Could you check a few things on this model? Use its own coordinates, in mm. Face numbers are marked on the shaded views. A direction names the side the tool comes from. Give positions to 0.01 mm unless a question says otherwise; leave off trailing zeros. Order: outer loops, then holes, each group sorted by start corner. A loop starts at its lowest first (then second) coordinate and runs counter-clockwise, first axis right, second up. Notation, with made-up numbers: (40, 80) -> (81, 80) arc R10 ccw to (81, 90) -> close; hole circle Ø5 at (12, 37). An arc over 180 degrees is marked (long way). One line per item, written item: value.
```python
from build123d import *

# Parameters (mm, degrees)
CUT_EXTRUDE_3_DEPTH = 1
SKETCH_5_R          = 1.5
CUT_EXTRUDE_4_DEPTH = 10
CHAMFER_1_SIZE      = 0.5
CHAMFER_2_SIZE      = 0.5


with BuildPart() as part:
    # 草图1 → 旋转2 (revolve)
    with BuildSketch(Plane.XY, mode=Mode.PRIVATE) as revolve_2_sk:
        Polygon((-23.267570956, 0), (-23.267570956, 4), (-8.267570956, 4), (-8.267570956, 5), (-2.267570956, 5), (-2.267570956, 6.5), (0.732429044, 6.5), (0.732429044, 5), (10.732429044, 5), (10.732429044, 4), (18.732429044, 4), (18.732429044, 0), align=None)
    revolve(revolve_2_sk.sketch.rotate(Axis((-82.03072058, 0, 0), (1, 0, 0)), 90), axis=Axis((-82.03072058, 0, 0), (1, 0, 0)))

    # 草图4 → 切除-拉伸3 (cut)
    with BuildSketch(Plane(origin=(0, 4, 0), x_dir=(1, 0, 0), z_dir=(0, 1, 0))):
        with BuildLine():
            Line((-19.767570956, 1), (-11.767570956, 1))
            ThreePointArc((-11.767570956, 1), (-10.767570956, 0), (-11.767570956, -1))
            Line((-11.767570956, -1), (-19.767570956, -1))
            ThreePointArc((-19.767570956, -1), (-20.767570956, 0), (-19.767570956, 1))
        make_face()
    extrude(amount=-CUT_EXTRUDE_3_DEPTH, mode=Mode.SUBTRACT)

    # 草图5 → 切除-拉伸4 (cut)
    with BuildSketch(Plane.ZY.offset(23.267570956)):
        Circle(SKETCH_5_R)
    extrude(amount=-CUT_EXTRUDE_4_DEPTH, mode=Mode.SUBTRACT)

    # 倒角1
    chamfer_1_edges = [part.edges().sort_by_distance(p)[0] for p in [
        (-23.267570956, 0, -4),
    ]]
    chamfer(chamfer_1_edges, length=CHAMFER_1_SIZE)

    # 倒角2
    chamfer_2_edges = [part.edges().sort_by_distance(p)[0] for p in [
        (18.732429044, 0, -4),
    ]]
    chamfer(chamfer_2_edges, length=CHAMFER_2_SIZE)


solid = part.part
```
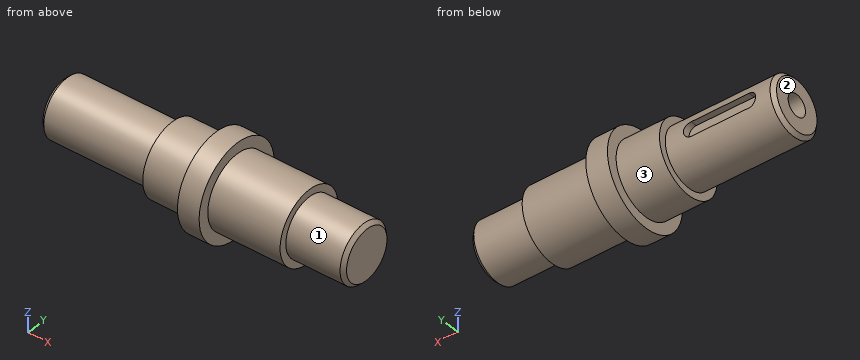
1) For P1, Ø2, axis at y = 4.5, z = -0.5, coming from the -X side; P2, Ø2.5, axis at y = 0, z = 0, coming from the -X side; P3, Ø0.6, axis at x = -13.5, z = -0.5, coming from the +Y side, each with a flat end and sliding along its axis, tell me the tip position at first contact or that it passes through.
Answer below:
P1: stops at x = -23.24
P2: stops at x = -13.27
P3: stops at y = 3
2) If I drill on line 1 along Y through (x, z) = (-17, 0); line 2 along X through (y, z) = (-0.5, 0.75); line 3 along X through (y, z) = (-6, 0.25), over which ranges is the centre line in solid material (lowest first)?
Answer below:
line 1: y = -4 to -1.5, 1.5 to 3
line 2: x = -13.27 to 18.73
line 3: x = -2.27 to 0.73
3) For the marked faces 1, 2 and 3, which set-ups out of +Z, -Z, +X, -X, +Y, -Y let a thin tool reach every point of the face, with its end or its side?
Answer below:
face 1: +X
face 2: +Z, -Z, -X, +Y, -Y
face 3: -X
4) Suppose I cut it at D-D, the plane x = -3. Write out the boundary of the cut face in (y, z).
Answer below:
outline: circle Ø10 at (0, 0)
5) Suppose I cut it at B-B, the plane y = 0. Write out the boundary of the cut face in (x, z), then the cut area to 4 significant figures.
Answer below:
outline: (-23.27, -3.5) -> (-22.77, -4) -> (-8.27, -4) -> (-8.27, -5) -> (-2.27, -5) -> (-2.27, -6.5) -> (0.73, -6.5) -> (0.73, -5) -> (10.73, -5) -> (10.73, -4) -> (18.23, -4) -> (18.73, -3.5) -> (18.73, 3.5) -> (18.23, 4) -> (10.73, 4) -> (10.73, 5) -> (0.73, 5) -> (0.73, 6.5) -> (-2.27, 6.5) -> (-2.27, 5) -> (-8.27, 5) -> (-8.27, 4) -> (-22.77, 4) -> (-23.27, 3.5) -> (-23.27, 1.5) -> (-13.27, 1.5) -> (-13.27, -1.5) -> (-23.27, -1.5) -> close
area: 352.5 mm2
6) Suppose I cut it at C-C, the plane x = 14. Write out the boundary of the cut face in (y, z), then the cut area to 3 significant figures.
Answer below:
outline: circle Ø8 at (0, 0)
area: 50.3 mm2
